For this review, take the finished solid that the model builds, in its own axes (mm). Face numbers are marked on the shaded views. A direction names the side the tool comes from. Round coordinates to 2 decimals unless told otherwise and drop trailing zeros. Order: outer loops, then holes, each group sorted by start corner. A loop starts at its lowest first (then second) coordinate and runs counter-clockwise, first axis right, second up. Notation, with made-up numbers: M -39.5,46 L -18.5,46 A10 cw -18.5,62 Z; hole C 29.5,-39 d6. An arc over 180 degrees is marked long. Answer as a JSON object with one key per item and string values.
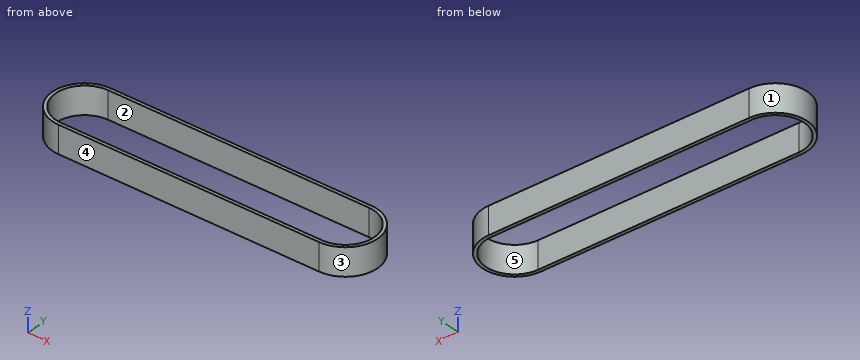
from build123d import *

# Parameters (mm, degrees)
EXTRUDE_THIN1_DEPTH = 12.5


with BuildPart() as part:
    # Sketch2 → Extrude-Thin1 (new, symmetric)
    with BuildSketch(Plane.XY):
        with BuildLine():
            Line((-235, 29.28), (0, 29.28))
            ThreePointArc((0, 29.28), (29.28, 0), (0, -29.28))
            Line((0, -29.28), (-235, -29.28))
            ThreePointArc((-235, -29.28), (-264.28, 0), (-235, 29.28))
        make_face()
        with BuildLine():
            Line((-235, 26.28), (0, 26.28))
            ThreePointArc((0, 26.28), (26.28, 0), (0, -26.28))
            Line((0, -26.28), (-235, -26.28))
            ThreePointArc((-235, -26.28), (-261.28, 0), (-235, 26.28))
        make_face(mode=Mode.SUBTRACT)
    extrude(amount=EXTRUDE_THIN1_DEPTH, both=True)


solid = part.part
1) Add section A-A on x = -229.5. State the section outline as (y, z) points, and give its area (3 significant figures).
Geometry check:
{"outline": "M -29.28,-12.5 L -26.28,-12.5 L -26.28,12.5 L -29.28,12.5 Z; M 26.28,-12.5 L 29.28,-12.5 L 29.28,12.5 L 26.28,12.5 Z", "area": "150 mm²"}
2) For L1, parallel to Y at x = -124.5, z = 5.25; L2, parallel to X at y = 0, z = 4.75; L3, parallel to X at y = -5.5, z = 2.25, list the stretches that pass through material, from the lowest coordinate up.
Geometry check:
{"L1": "y = -29.28 to -26.28, 26.28 to 29.28", "L2": "x = -264.28 to -261.28, 26.28 to 29.28", "L3": "x = -263.76 to -260.7, 25.7 to 28.76"}
3) Add section B-B on y = 0. State the section outline as (x, z) points.
Geometry check:
{"outline": "M -264.28,-12.5 L -261.28,-12.5 L -261.28,12.5 L -264.28,12.5 Z; M 26.28,-12.5 L 29.28,-12.5 L 29.28,12.5 L 26.28,12.5 Z"}
4) Machinability: for the marked faces 1 and 2, which of the approach directions +Z, -Z, +X, -X, +Y, -Y give a long, thin tool a straight path to every point of the face, cutting with its end or side? Answer none if there is none.
Geometry check:
{"face 1": "+Z, -Z, -X", "face 2": "+Z, -Z"}
5) Add section C-C on z = -9. State the section outline as (x, y) points, and give its area (3 significant figures).
Geometry check:
{"outline": "M -235,-29.28 L 0,-29.28 A29.28 ccw 0,29.28 L -235,29.28 A29.28 ccw Z; hole M -235,-26.28 L 0,-26.28 A26.28 ccw 0,26.28 L -235,26.28 A26.28 ccw Z", "area": "1,930 mm²"}
6) Mouldability with a two-part tool opening along Y and no side actions: class the marked faces 3, 4 and 5 as +Y half, -Y half, draft (parallel to the pull), parting line (faces both ways), or undercut.
Geometry check:
{"face 3": "parting line", "face 4": "-Y half", "face 5": "undercut"}
7) Insertion check: P1, Ø3, axis at y = 15.5, z = 5.5, coming from the -X side; P2, Ø6, axis at y = 4, z = 8.5, coming from the -X side; P3, Ø8, axis at y = -7, z = 1, coming from the -X side. Each pin has a flat end and moves straight along its axis. Give the tip position at first contact, or say it passes through.
Geometry check:
{"P1": "stops at x = -260.72", "P2": "stops at x = -264.26", "P3": "stops at x = -264.13"}
